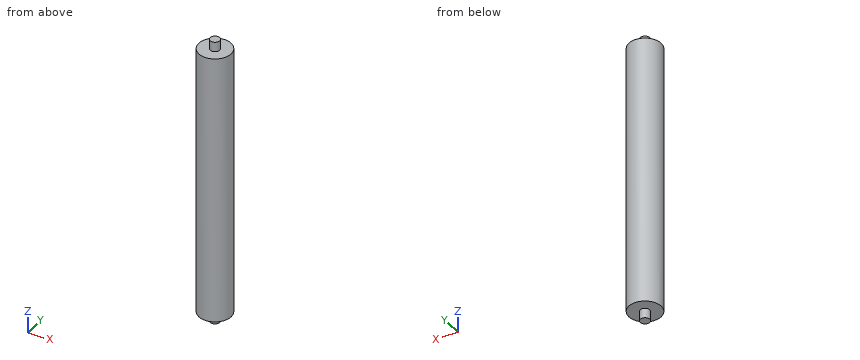
```python
from build123d import *

# Parameters (mm, degrees)
SKETCH_1_R      = 25
EXTRUDE_1_DEPTH = 420
SKETCH_2_R      = 7.5
EXTRUDE_2_DEPTH = 15
EXTRUDE_START   = 15
SKETCH_3_R      = 7.5
EXTRUDE_3_DEPTH = 15


with BuildPart() as part:
    # 草图1 → 凸台-拉伸1 (new body)
    with BuildSketch(Plane.XY):
        Circle(SKETCH_1_R)
    extrude(amount=EXTRUDE_1_DEPTH)

    # 草图2 → 凸台-拉伸2 (add)
    with BuildSketch(Plane.XY.offset(420)):
        Circle(SKETCH_2_R)
    extrude(amount=EXTRUDE_2_DEPTH)

    # 草图3 → 凸台-拉伸3 (add)
    with BuildSketch(Plane(origin=(0, 0, 0), x_dir=(-1, 0, 0), z_dir=(0, 0, -1)).offset(EXTRUDE_START)):
        with Locations(Location((0, 0, 0), (0, 0, 180))):
            Circle(SKETCH_3_R)
    extrude(amount=-EXTRUDE_3_DEPTH)


solid = part.part
```
Work out the finished part from the listing and answer in its coordinate system (mm). Coordinates: 2 decimals unless noted, no trailing zeros. Write each loop counter-clockwise with the first axis right and the second up, starting at its lowest first coordinate (ties: lowest second). Pieces come first, ordered by that corner, then holes.
Q1. Find the intervals of material crossed by line 1 (Z direction, x = -13, y = 5); line 2 (X direction, y = 1.5, z = 290.5); line 3 (X direction, y = -3, z = 91), in increasing order.
Q2. Each of these flat-tipped pins is pushed along its axis until it touches: pin 1 Ø2 at (x, z) = (-6, 373.5) entering from -Y; pin 2 Ø4 at (x, y) = (18, -11.5) entering from -Z; pin 3 Ø4 at (x, y) = (16.5, 1) entering from +Z; pin 4 Ø25 at (x, y) = (-5, 11.5) entering from -Z. Where does it stop, or does it pass through?
Q3. A cutting plane is placed at C-C, the plane z = 390. Give the vertices of the cut face in (x, y).
Q4. A cutting plane is placed at A-A, the plane y = 0. Give the vertices of the cut face in (x, z), then the cut area to 4 significant figures.
Q5. A cutting plane is placed at D-D, the plane y = 18.5. Give the vertices of the cut face in (x, z), then the cut area to 3 significant figures.
Findings below:
1. line 1: z = 0 to 420
1. line 2: x = -24.95 to 24.95
1. line 3: x = -24.82 to 24.82
2. pin 1: stops at y = -24.49
2. pin 2: stops at z = 0
2. pin 3: stops at z = 420
2. pin 4: stops at z = -15
3. outline: circle Ø50 at (0, 0)
4. outline: (-25, 0) - (-7.5, 0) - (-7.5, -15) - (7.5, -15) - (7.5, 0) - (25, 0) - (25, 420) - (7.5, 420) - (7.5, 435) - (-7.5, 435) - (-7.5, 420) - (-25, 420) - close
4. area: 21,450 mm2
5. outline: (-16.82, 0) - (16.82, 0) - (16.82, 420) - (-16.82, 420) - close
5. area: 14,100 mm2
